from build123d import *

# Parameters (mm, degrees)
SKETCH1_W           = 40
SKETCH1_H           = 80
SKETCH1_R           = 5
BOSS_EXTRUDE1_DEPTH = 14


with BuildPart() as part:
    # Sketch1 → Boss-Extrude1 (new body)
    with BuildSketch(Plane.XY):
        with Locations((20, 40)):
            Rectangle(SKETCH1_W, SKETCH1_H)
        with Locations((20, 40)):
            Circle(SKETCH1_R, mode=Mode.SUBTRACT)
    extrude(amount=BOSS_EXTRUDE1_DEPTH)


solid = part.part
Work out the finished part from the listing and answer in its coordinate system (mm). Give positions to 0.01 mm unless a question says otherwise; leave off trailing zeros. Order: outer loops, then holes, each group sorted by start corner. A loop starts at its lowest first (then second) coordinate and runs counter-clockwise, first axis right, second up. Notation, with made-up numbers: (61, 50) -> (120, 50) arc R16 ccw to (120, 59) -> close; hole circle Ø7 at (19.5, 83.25). An arc over 180 degrees is marked (long way). Answer as a JSON object with one key per item and string values. Group by question number.
1. Section C-C on z = 2 is taken. Determine the outline of the cut face in (x, y).
2. Consider line 1 along Y through (x, z) = (20, 9); line 2 along X through (y, z) = (38.5, 13.25); line 3 along Y through (x, z) = (21, 9.75). Determine where each line is inside the solid, lowest interval first. Write a range as [from, to].
3. Section A-A on y = 40 is taken. Determine the outline of the cut face in (x, z).
4. A flat-ended cylindrical pin translates along its axis: pin 1 Ø9 at (x, y) = (20, 40) entering from -Z. Find the tip coordinate at first contact, or state that the pin passes through.
5. Section B-B on x = 20 is taken. Determine the outline of the cut face in (y, z).
6. The mould has two halves that part along X. Classify faces 1 (the flat face through (0, 39, 7)), 2 (the flat face through (20, 0, 7)), 3 (the cylindrical face through (19.349, 44.957, 6.902)): released by +X, released by -X, zero draft, split by the parting line, or undercut.
Result sheet:
{
 "1": {"outline": "(0, 0) -> (40, 0) -> (40, 80) -> (0, 80) -> close; hole circle Ø10 at (20, 40)"},
 "2": {"line 1": "y = [0, 35], [45, 80]", "line 2": "x = [0, 15.23], [24.77, 40]", "line 3": "y = [0, 35.1], [44.9, 80]"},
 "3": {"outline": "(0, 0) -> (15, 0) -> (15, 14) -> (0, 14) -> close; (25, 0) -> (40, 0) -> (40, 14) -> (25, 14) -> close"},
 "4": {"pin 1": "passes through"},
 "5": {"outline": "(0, 0) -> (35, 0) -> (35, 14) -> (0, 14) -> close; (45, 0) -> (80, 0) -> (80, 14) -> (45, 14) -> close"},
 "6": {"face 1": "released by -X", "face 2": "zero draft", "face 3": "undercut"}
}
